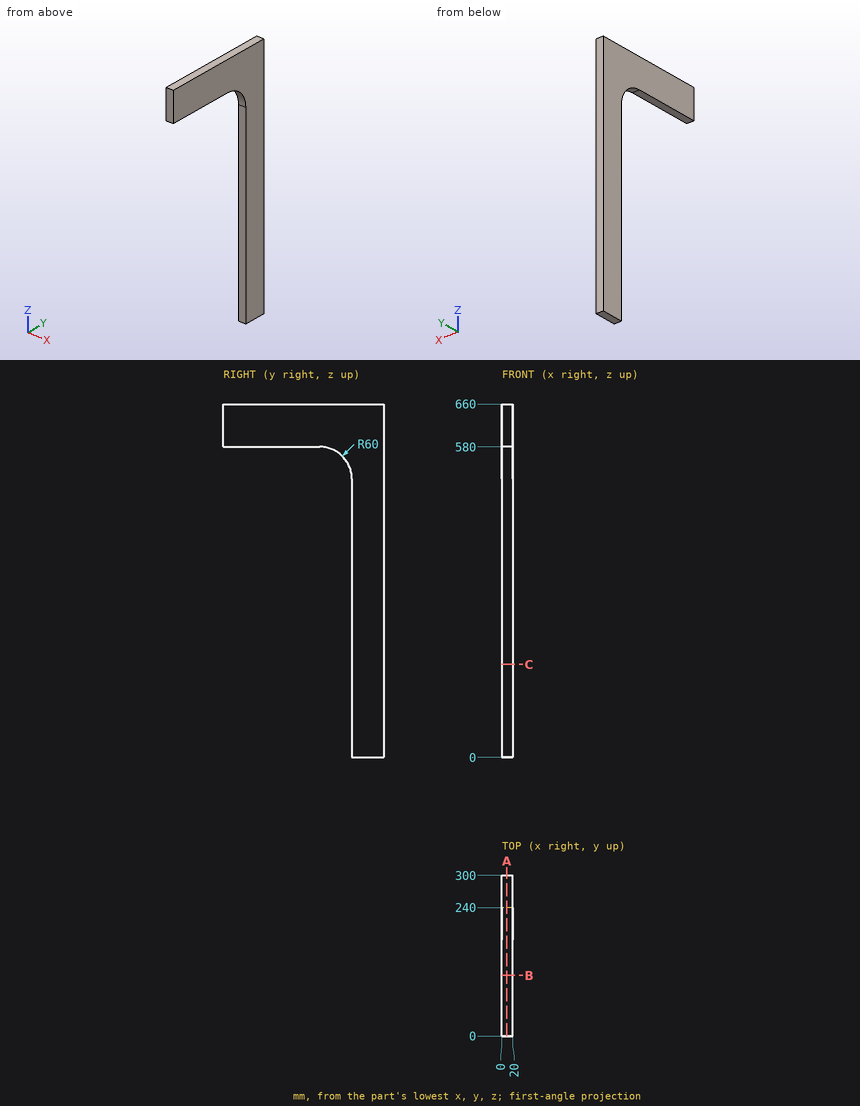
The drawing under review shows one solid part. Ordinate dimensions are in mm from its lowest x, y, z. Round coordinates to 2 decimals unless told otherwise and drop trailing zeros. Loops run counter-clockwise (first coordinate to the right, second up) from the corner with the lowest first, then second, coordinate; pieces in that order, holes last. Notation, with made-up numbers: M 56.25,76 L 97.25,76 A22 ccw 97.25,104 Z; hole C 80.25,70.25 d6. An arc over 180 degrees is marked long. Answer as CSV lines item,"result". Start each with the question number.
Item 1: Consider section B-B (y = 113). Write out the cut boundary in (x, z), then the cut area to 3 significant figures.
Item 2: Wall thickness on line 1 (Z direction, x = 5, y = 21); line 2 (Y direction, x = 16.5, z = 131); line 3 (Z direction, x = 8.25, y = 189): over which ranges is each line inside the solid? List them lowest first. Write a range as [from, to].
Item 3: Consider section A-A (x = 9). Write out the cut boundary in (y, z).
Item 4: Consider section C-C (z = 173.5). Write out the cut boundary in (x, y), then the cut area to 3 significant figures.
Item 5: Insertion check: P1, Ø2, axis at x = 5.5, y = 43, coming from the -Z side; P2, Ø6, axis at x = 10.5, z = 372.5, coming from the -Y side. Each pin has a flat end and moves straight along its axis. Give the tip position at first contact, or say it passes through.
Answer:
1,outline,"M 0,580 L 20,580 L 20,660 L 0,660 Z"
1,area,"1,600 mm^2"
2,line 1,"z = [580, 660]"
2,line 2,"y = [240, 300]"
2,line 3,"z = [579.32, 660]"
3,outline,"M 0,580 L 180,580 A60 cw 240,520 L 240,0 L 300,0 L 300,660 L 0,660 Z"
4,outline,"M 0,240 L 20,240 L 20,300 L 0,300 Z"
4,area,"1,200 mm^2"
5,P1,"stops at z = 580"
5,P2,"stops at y = 240"
